Design review of the part built by this model. Coordinates are the model's own, in mm. A direction names the side the tool comes from. Give positions to 0.01 mm unless a question says otherwise; leave off trailing zeros. Order: outer loops, then holes, each group sorted by start corner. A loop starts at its lowest first (then second) coordinate and runs counter-clockwise, first axis right, second up. Notation, with made-up numbers: (32.25, 22.5) -> (70.25, 22.5) arc R11 cw to (70.25, 31.5) -> close; hole circle Ø8 at (14, -18). An arc over 180 degrees is marked (long way). Return JSON: item names as keys, results as strings.
```python
from build123d import *

# Parameters (mm, degrees)
SKETCH1_R           = 2.5
BOSS_EXTRUDE1_DEPTH = 25
CHAMFER1_SIZE       = 0.3
SKETCH3_W           = 4.032252552
SKETCH3_H           = 0.6
CUT_EXTRUDE2_DEPTH  = 6


with BuildPart() as part:
    # Sketch1 → Boss-Extrude1 (new body)
    with BuildSketch(Plane(origin=(0, 0, 0), x_dir=(1, 0, 0), z_dir=(0, 1, 0))):
        with Locations(Location((0, 0, 0), (0, 0, 270))):
            Circle(SKETCH1_R)
    extrude(amount=BOSS_EXTRUDE1_DEPTH)

    # Chamfer1
    chamfer1_edges = [part.edges().sort_by_distance(p)[0] for p in [
        (0, 0, -2.5),
        (0, 25, -2.5),
    ]]
    chamfer(chamfer1_edges, length=CHAMFER1_SIZE)

    # Sketch3 → Cut-Extrude2 (cut)
    with BuildSketch(Plane.XZ):
        with Locations((0, 2.5)):
            Rectangle(SKETCH3_W, SKETCH3_H)
    extrude(amount=-CUT_EXTRUDE2_DEPTH, mode=Mode.SUBTRACT)


solid = part.part
```
Item 1: Machinability: for faces 1 (the face through (0, 25, 0)), 2 (the face through (0, 3, 2.2)), which of the approach directions +Z, -Z, +X, -X, +Y, -Y give a long, thin tool a straight path to every point of the face, cutting with its end or side? Answer none if there is none.
Result set:
{"face 1": "+Z, -Z, +X, -X, +Y", "face 2": "+Z, +X, -X, -Y"}
Item 2: Wall thickness on L1, parallel to Z at x = 0, y = 3.25; L2, parallel to X at y = 4.75, z = 0.45; L3, parallel to X at y = 18, z = 0.5: over which ranges is each line inside the solid? List them lowest first. Write a range as [from, to].
Result set:
{"L1": "z = [-2.5, 2.2]", "L2": "x = [-2.46, 2.46]", "L3": "x = [-2.45, 2.45]"}
Item 3: Add section B-B (y = 3.75). Give the boundary of the cut face in (x, z), plus the area to 3 significant figures.
Result set:
{"outline": "(-1.19, 2.2) arc R2.5 ccw (long way) to (1.19, 2.2) -> close", "area": "19.2 mm^2"}
Item 4: Add section A-A (y = 17.5). Give the boundary of the cut face in (x, z), plus the area to 3 significant figures.
Result set:
{"outline": "circle Ø5 at (0, 0)", "area": "19.6 mm^2"}
Item 5: For pin 1 (1.5 mm diameter, centred on y = 14.5, z = 1.5, fed in from -X); pin 2 (1.2 mm diameter, centred on x = 0.5, y = 3.5, fed in from +Z); pin 3 (1 mm diameter, centred on x = 1.5, y = 17.5, fed in from -Z); pin 4 (3 mm diameter, centred on x = -1.5, y = 22, fed in from -Z), all flat-tipped, find the tip position at first contact; note any pin that passes through.
Result set:
{"pin 1": "stops at x = -2.38", "pin 2": "stops at z = 2.2", "pin 3": "stops at z = -2.29", "pin 4": "stops at z = -2.5"}
